Could you check a few things on this model? Use its own coordinates, in mm. A direction names the side the tool comes from. Coordinates: 2 decimals unless noted, no trailing zeros. Order: outer loops, then holes, each group sorted by start corner. A loop starts at its lowest first (then second) coordinate and runs counter-clockwise, first axis right, second up.
```python
from build123d import *

# Parameters (mm, degrees)
SKETCH_1_R           = 2.5
SKETCH_1_R_2         = 55
EXTRUDE_1_DEPTH      = 6
SKETCH_4_W           = 30
SKETCH_4_H           = 120
EXTRUDE_3_DEPTH      = 6
SKETCH_5_R           = 4.5
CUT_EXTRUDE_1_DEPTH  = 6
EXTRUDE_4_DEPTH      = 3
EXTRUDE_4_DEPTH_BACK = 3


with BuildPart() as part:
    # 草图1 → 凸台-拉伸1 (new body)
    with BuildSketch(Plane.XY):
        Polygon((0, 0), (30, 0), (180, 30), (180, 150), (0, 150), align=None)
        with Locations((165.5, 135.5)):
            Circle(SKETCH_1_R, mode=Mode.SUBTRACT)
        with Locations((68.5, 135.5)):
            Circle(SKETCH_1_R, mode=Mode.SUBTRACT)
        with Locations((165.5, 38.5)):
            Circle(SKETCH_1_R, mode=Mode.SUBTRACT)
        with Locations((68.5, 38.5)):
            Circle(SKETCH_1_R, mode=Mode.SUBTRACT)
        with Locations((117, 87)):
            Circle(SKETCH_1_R_2, mode=Mode.SUBTRACT)
    extrude(amount=EXTRUDE_1_DEPTH)

    # 草图4 → 凸台-拉伸3 (add)
    with BuildSketch(Plane.XZ):
        with Locations((15, 3)):
            Rectangle(SKETCH_4_W, SKETCH_4_H)
    extrude(amount=EXTRUDE_3_DEPTH)

    # 草图5 → 切除-拉伸1 (cut)
    with BuildSketch(Plane(origin=(0, 0, 0), x_dir=(1, 0, 0), z_dir=(0, 1, 0))):
        with Locations(Location((13, 47, 0), (0, 0, 270))):
            Circle(SKETCH_5_R)
        with Locations(Location((13, -53, 0), (0, 0, 270))):
            Circle(SKETCH_5_R)
    extrude(amount=-CUT_EXTRUDE_1_DEPTH, mode=Mode.SUBTRACT)

    # 草图6 → 凸台-拉伸4 (add, two sides: drawn at the far end of the back side and taken through both)
    with BuildSketch(Plane.ZY.offset(-15).offset(-EXTRUDE_4_DEPTH_BACK)):
        Polygon((0, 90), (-30, 0), (0, 0), align=None)
        Polygon((6, 0), (6, 90), (36, 0), align=None)
    extrude(amount=EXTRUDE_4_DEPTH + EXTRUDE_4_DEPTH_BACK)


solid = part.part
```
Item 1: Suppose I cut it at A-A (z = -47). List the corners of the cut face in (x, y) for me.
Item 2: Suppose I cut it at C-C (y = 43.5). List the corners of the cut face in (x, z) for me, and give its area (3 significant figures).
Item 3: Which directions (+Z, -Z, +X, -X, +Y, -Y) give clear straight access to the entire face, cutting with the end or side of a thin tool? Please do faces 1 (the face through (11, 0, -28)), 2 (the face through (18, 26, 15)), 3 (the face through (11, 0, 35)).
Item 4: Suppose I cut it at B-B (x = 97.5). List the corners of the cut face in (y, z) for me, and give its area (3 significant figures).
Item 5: For pin 1 Ø3 at (x, y) = (165.5, 38.5) entering from -Z; pin 2 Ø8 at (x, y) = (68.5, 38.5) entering from +Z; pin 3 Ø5 at (y, z) = (37, 11) entering from -X; pin 4 Ø9 at (x, z) = (8.5, -40) entering from +Y, each with a flat end and sliding along its axis, tell me the tip position at first contact or that it passes through.
Item 6: Suppose I cut it at D-D (x = 27). List the corners of the cut face in (y, z) for me.
Item 7: Thinking about a two-plate mould opening in X: for faces 4 (the face through (0, 38, 3)), 5 (the face through (30, -3, 2)), 6 (the face through (14.352, -2.958, 57.292)), which applies, +X half, -X half, draft (parallel to the pull), parting line (faces both ways), or undercut?
Item 8: I need wall thicknesses on line 1 (X direction, y = 135.5, z = 2.75); line 2 (X direction, y = -1.3, z = 53); line 3 (Z direction, x = 18, y = 138.5). Which ranges of each line are inside material? Lowest first, please.
Geometry results:
1. outline: (0, -6) - (8.5, -6) - (8.5, 0) - (0, 0) - close; (17.5, -6) - (30, -6) - (30, 0) - (17.5, 0) - close
2. outline: (0, 0) - (12, 0) - (12, -15.5) - (18, -15.5) - (18, 0) - (83.34, 0) - (83.34, 6) - (18, 6) - (18, 21.5) - (12, 21.5) - (12, 6) - (0, 6) - close; (150.66, 0) - (180, 0) - (180, 6) - (150.66, 6) - close
2. area: 862 mm2
3. face 1: -Z, +Y
3. face 2: +Z, +X, +Y
3. face 3: +Z, +Y
4. outline: (13.5, 0) - (35.57, 0) - (35.57, 6) - (13.5, 6) - close; (138.43, 0) - (150, 0) - (150, 6) - (138.43, 6) - close
4. area: 202 mm2
5. pin 1: passes through
5. pin 2: stops at z = 6
5. pin 3: stops at x = 12
5. pin 4: stops at y = 0
6. outline: (-6, -57) - (0, -57) - (0, 0) - (150, 0) - (150, 6) - (0, 6) - (0, 63) - (-6, 63) - close
7. face 4: -X half
7. face 5: +X half
7. face 6: undercut
8. line 1: x = 0 to 66, 71 to 91.06, 142.94 to 163, 168 to 180
8. line 2: x = 0 to 8.5, 17.5 to 30
8. line 3: z = 0 to 6
